Here's how the part is built. I have some questions about the finished solid (model axes, mm). Face numbers are marked on the shaded views. A direction names the side the tool comes from. Round coordinates to 2 decimals unless told otherwise and drop trailing zeros. Write each loop counter-clockwise with the first axis right and the second up, starting at its lowest first coordinate (ties: lowest second). Pieces come first, ordered by that corner, then holes. Notation, with made-up numbers: (2.5, 83) - (53.5, 83) arc R33 cw to (53.5, 116) - close; hole circle Ø4 at (14, 83.25). An arc over 180 degrees is marked (long way). One line per item, written item: value. Start each with the question number.
Item 1: Imagine slicing it at B-B, the plane x = 23. Please give me the cut outline in (y, z).
Item 2: If I drill on line 1 (X direction, y = 5, z = 0); line 2 (Y direction, x = 46, z = -16.5); line 3 (X direction, y = -12.5, z = 13.5), over which ranges is the centre line in solid material (lowest first)?
Item 3: Imagine slicing it at C-C, the plane x = 125. Please give me the cut outline in (y, z) (1 decimal).
Item 4: Imagine slicing it at A-A, the plane x = 74. Please give me the cut outline in (y, z).
Item 5: For the marked faces 1, 2, 3, 4 and 5, which set-ups out of +Z, -Z, +X, -X, +Y, -Y let a thin tool reach every point of the face, with its end or its side?
Item 6: For P1, Ø8, axis at x = 62, z = -12.5, coming from the -Y side; P2, Ø3, axis at y = 6, z = -16, coming from the -X side; P3, Ø4, axis at x = 99.5, z = 10.5, coming from the -Y side, each with a flat end and sliding along its axis, tell me the tip position at first contact or that it passes through.
```python
from build123d import *

# Parameters (mm, degrees)
CHAMFER1_SIZE       = 1.524
BOSS_EXTRUDE1_DEPTH = 18.923
FILLET1_R           = 0.762
SKETCH3_R           = 1.98435
CUT_EXTRUDE1_DEPTH  = 25


with BuildPart() as part:
    # Sketch1 → Revolve1 (revolve)
    with BuildSketch(Plane.XY, mode=Mode.PRIVATE) as revolve1_sk:
        Polygon((0, 0), (0, 14.1605), (31.75, 14.1605), (31.75, 12.065), (38.1, 12.065), (38.1, 19.05), (75.692, 19.05), (75.692, 15.5575), (136.144, 15.5575), (136.144, 0), align=None)
    revolve(revolve1_sk.sketch.rotate(Axis((0, 0, 0), (1, 0, 0)), 90), axis=Axis((0, 0, 0), (1, 0, 0)))

    # Chamfer1
    chamfer1_edges = [part.edges().sort_by_distance(p)[0] for p in [
        (0, 0, -14.1605),
        (136.144, 0, -15.5575),
    ]]
    chamfer(chamfer1_edges, length=CHAMFER1_SIZE)

    # Sketch2 → Boss-Extrude1 (add)
    with BuildSketch(Plane(origin=(75.692, 0, 0), x_dir=(0, 0, -1), z_dir=(1, 0, 0))):
        Polygon((0, 21.997045256), (-19.05, 10.998522628), (-19.05, -10.998522628), (0, -21.997045256), (19.05, -10.998522628), (19.05, 10.998522628), align=None)
    extrude(amount=-BOSS_EXTRUDE1_DEPTH)

    # Fillet1
    fillet1_edges = [part.edges().sort_by_distance(p)[0] for p in [
        (38.1, 0, -12.065),
        (31.75, 0, -12.065),
    ]]
    fillet(fillet1_edges, radius=FILLET1_R)

    # Sketch3 → Cut-Extrude1 (cut, symmetric)
    with BuildSketch(Plane(origin=(0, 0, 0), x_dir=(1, 0, 0), z_dir=(0, 1, 0))):
        with Locations(Location((131.318, 0, 0), (0, 0, 270))):
            Circle(SKETCH3_R)
    extrude(amount=CUT_EXTRUDE1_DEPTH, both=True, mode=Mode.SUBTRACT)


solid = part.part
```
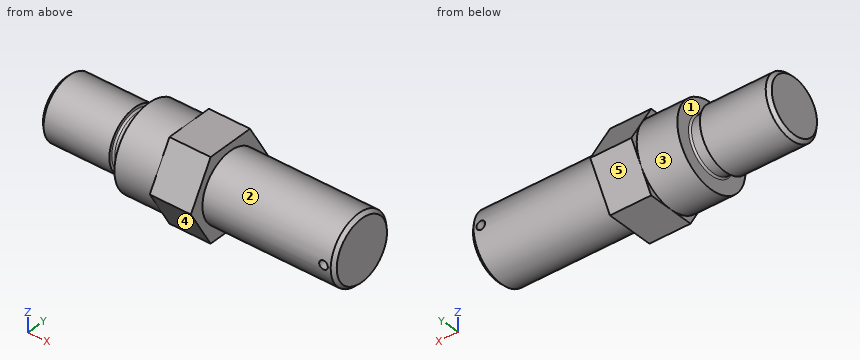
Values follow:
1. outline: circle Ø28.32 at (0, 0)
2. line 1: x = 0 to 129.33, 133.3 to 136.14
2. line 2: y = -9.52 to 9.52
2. line 3: x = 38.1 to 75.69
3. outline: circle Ø31.1 at (0, 0)
4. outline: (-22, 0) - (-11, -19.05) - (11, -19.05) - (22, 0) - (11, 19.05) - (-11, 19.05) - close
5. face 1: none
5. face 2: +X
5. face 3: -X
5. face 4: -Z, +X, -X, -Y
5. face 5: -Z, +X, -X, +Y
6. P1: stops at y = -17.09
6. P2: stops at x = 38.1
6. P3: stops at y = -13.03
